Could you check a few things on this drawing? It's one solid part, dimensions in mm from its lowest x, y, z. A direction names the side the tool comes from. Give positions to 0.01 mm unless a question says otherwise; leave off trailing zeros. Order: outer loops, then holes, each group sorted by start corner. A loop starts at its lowest first (then second) coordinate and runs counter-clockwise, first axis right, second up. Notation, with made-up numbers: (43, 41) -> (66, 41) arc R24 cw to (66, 77) -> close; hole circle Ø4 at (83.25, -31). An arc over 180 degrees is marked (long way). Answer as a JSON object with one key per item and string values.
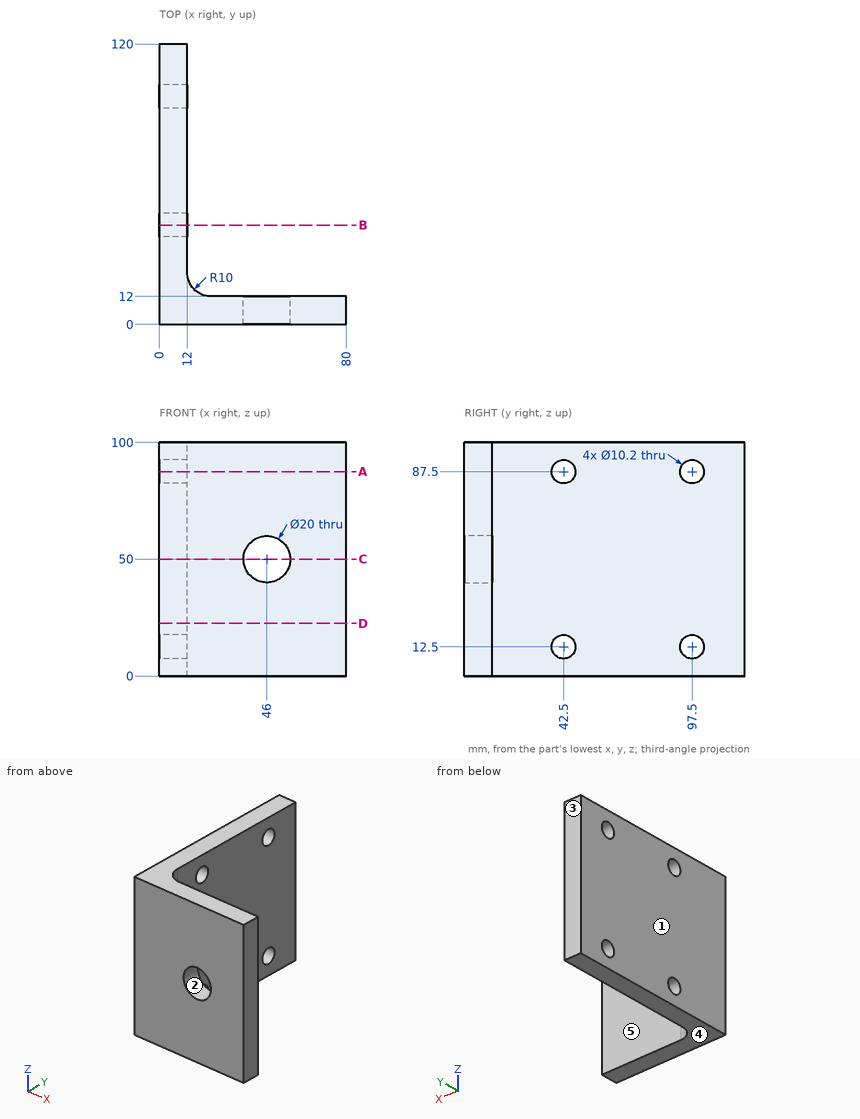
1. If we section it at A-A on z = 87.5: Please give me the cut outline in (x, y).
Worked answers:
{"outline": "(0, 0) -> (80, 0) -> (80, 12) -> (22, 12) arc R10 cw to (12, 22) -> (12, 37.4) -> (0, 37.4) -> close; (0, 47.6) -> (12, 47.6) -> (12, 92.4) -> (0, 92.4) -> close; (0, 102.6) -> (12, 102.6) -> (12, 120) -> (0, 120) -> close"}
2. If we mould it in two halves opening along X, with no side actions, what happens to the marked faces 1, 2 and 3? For each: +X half, -X half, draft (parallel to the pull), parting line (faces both ways), or undercut.
Worked answers:
{"face 1": "-X half", "face 2": "undercut", "face 3": "draft"}
3. For the marked faces 4 and 5, which set-ups out of +Z, -Z, +X, -X, +Y, -Y let a thin tool reach every point of the face, with its end or its side?
Worked answers:
{"face 4": "-Z, +X, -X, +Y, -Y", "face 5": "+Z, -Z, +X, +Y"}
4. If we section it at B-B on y = 42.5: Please give me the cut outline in (x, z), then the cut area to 3 significant figures.
Worked answers:
{"outline": "(0, 0) -> (12, 0) -> (12, 7.4) -> (0, 7.4) -> close; (0, 17.6) -> (12, 17.6) -> (12, 82.4) -> (0, 82.4) -> close; (0, 92.6) -> (12, 92.6) -> (12, 100) -> (0, 100) -> close", "area": "955 mm²"}
5. If we section it at D-D on z = 22.5: Please give me the cut outline in (x, y), then the cut area to 3 significant figures.
Worked answers:
{"outline": "(0, 0) -> (80, 0) -> (80, 12) -> (22, 12) arc R10 cw to (12, 22) -> (12, 120) -> (0, 120) -> close", "area": "2,280 mm²"}
6. If we section it at C-C on z = 50: Please give me the cut outline in (x, y), then the cut area to 3 significant figures.
Worked answers:
{"outline": "(0, 0) -> (36, 0) -> (36, 12) -> (22, 12) arc R10 cw to (12, 22) -> (12, 120) -> (0, 120) -> close; (56, 0) -> (80, 0) -> (80, 12) -> (56, 12) -> close", "area": "2,040 mm²"}
7. Will these pins go through, and if not, where does the flat tip stop? pin 1 Ø2 at (y, z) = (52, 84) entering from +X; pin 2 Ø4 at (x, z) = (36, 55.5) entering from +Y.
Worked answers:
{"pin 1": "x = 12", "pin 2": "y = 12"}
8. Please list where these lines run through material, in increasing order: L1, parallel to Y at x = 3.75, z = 12.5; L2, parallel to Z at x = 9, y = 97; L3, parallel to Y at x = 66, z = 77.5.
Worked answers:
{"L1": "0 to 37.4, 47.6 to 92.4, 102.6 to 120", "L2": "0 to 7.42, 17.58 to 82.42, 92.58 to 100", "L3": "0 to 12"}
